```python
from build123d import *

# Parameters (mm, degrees)
SKETCH_1_R          = 52.5
SKETCH_1_R_2        = 16
SKETCH_1_R_3        = 3
EXTRUDE_1_DEPTH     = 10
SKETCH_2_R          = 24
SKETCH_2_R_2        = 16
EXTRUDE_2_DEPTH     = 20
CUT_EXTRUDE_START   = -3
CUT_EXTRUDE_2_DEPTH = 3


with BuildPart() as part:
    # 草图1 → 凸台-拉伸1 (new body)
    with BuildSketch(Plane.XY):
        Circle(SKETCH_1_R)
        Circle(SKETCH_1_R_2, mode=Mode.SUBTRACT)
        with Locations((0, 40)):
            Circle(SKETCH_1_R_3, mode=Mode.SUBTRACT)
        with Locations((40, 0)):
            Circle(SKETCH_1_R_3, mode=Mode.SUBTRACT)
        with Locations((0, -40)):
            Circle(SKETCH_1_R_3, mode=Mode.SUBTRACT)
        with Locations((-40, 0)):
            Circle(SKETCH_1_R_3, mode=Mode.SUBTRACT)
    extrude(amount=EXTRUDE_1_DEPTH)

    # 草图2 → 凸台-拉伸2 (add)
    with BuildSketch(Plane.XY.offset(10)):
        Circle(SKETCH_2_R)
        Circle(SKETCH_2_R_2, mode=Mode.SUBTRACT)
    extrude(amount=EXTRUDE_2_DEPTH)

    # 草图3 → 切除-拉伸2 (cut)
    with BuildSketch(Plane.XY.offset(30).offset(CUT_EXTRUDE_START)):
        with BuildLine():
            Line((-4, 23.664319132), (-4, 15.491933385))
            ThreePointArc((-4, 15.491933385), (0, 16), (4, 15.491933385))
            Line((4, 15.491933385), (4, 23.664319132))
            ThreePointArc((4, 23.664319132), (0, 24), (-4, 23.664319132))
        make_face()
        with BuildLine():
            Line((13.904773406, 19.561627655), (8.126024025, 13.782878275))
            ThreePointArc((8.126024025, 13.782878275), (11.313708499, 11.313708499), (13.782878275, 8.126024025))
            Line((13.782878275, 8.126024025), (19.561627655, 13.904773406))
            ThreePointArc((19.561627655, 13.904773406), (16.970562748, 16.970562748), (13.904773406, 19.561627655))
        make_face()
        with BuildLine():
            Line((23.664319132, 4), (15.491933385, 4))
            ThreePointArc((15.491933385, 4), (16, 0), (15.491933385, -4))
            Line((15.491933385, -4), (23.664319132, -4))
            ThreePointArc((23.664319132, -4), (24, 0), (23.664319132, 4))
        make_face()
        with BuildLine():
            Line((19.561627655, -13.904773406), (13.782878275, -8.126024025))
            ThreePointArc((13.782878275, -8.126024025), (11.313708499, -11.313708499), (8.126024025, -13.782878275))
            Line((8.126024025, -13.782878275), (13.904773406, -19.561627655))
            ThreePointArc((13.904773406, -19.561627655), (16.970562748, -16.970562748), (19.561627655, -13.904773406))
        make_face()
        with BuildLine():
            Line((4, -23.664319132), (4, -15.491933385))
            ThreePointArc((4, -15.491933385), (0, -16), (-4, -15.491933385))
            Line((-4, -15.491933385), (-4, -23.664319132))
            ThreePointArc((-4, -23.664319132), (0, -24), (4, -23.664319132))
        make_face()
        with BuildLine():
            Line((-13.904773406, -19.561627655), (-8.126024025, -13.782878275))
            ThreePointArc((-8.126024025, -13.782878275), (-11.313708499, -11.313708499), (-13.782878275, -8.126024025))
            Line((-13.782878275, -8.126024025), (-19.561627655, -13.904773406))
            ThreePointArc((-19.561627655, -13.904773406), (-16.970562748, -16.970562748), (-13.904773406, -19.561627655))
        make_face()
        with BuildLine():
            Line((-23.664319132, -4), (-15.491933385, -4))
            ThreePointArc((-15.491933385, -4), (-16, 0), (-15.491933385, 4))
            Line((-15.491933385, 4), (-23.664319132, 4))
            ThreePointArc((-23.664319132, 4), (-24, 0), (-23.664319132, -4))
        make_face()
        with BuildLine():
            Line((-19.561627655, 13.904773406), (-13.782878275, 8.126024025))
            ThreePointArc((-13.782878275, 8.126024025), (-11.313708499, 11.313708499), (-8.126024025, 13.782878275))
            Line((-8.126024025, 13.782878275), (-13.904773406, 19.561627655))
            ThreePointArc((-13.904773406, 19.561627655), (-16.970562748, 16.970562748), (-19.561627655, 13.904773406))
        make_face()
    extrude(amount=CUT_EXTRUDE_2_DEPTH, mode=Mode.SUBTRACT)


solid = part.part
```
Part model, mm, in its own coordinate system. A direction names the side the tool comes from. Coordinates: 2 decimals unless noted, no trailing zeros. Loops run counter-clockwise (first coordinate to the right, second up) from the corner with the lowest first, then second, coordinate; pieces in that order, holes last. Notation, with made-up numbers: (5, 55) - (23, 55) arc R28 cw to (23, 81) - close; hole circle Ø6 at (-10, -1). An arc over 180 degrees is marked (long way). Write item = value, one per line. Start each with the question number.
Item 1: Cut at C-C, the plane z = 2.25. Give the cut face in (x, y).
Item 2: Wall check: L1, parallel to Y at x = 0, z = 2.5; L2, parallel to Y at x = 0, z = 12.75; L3, parallel to Z at x = 17.5, y = 34.5. Give the ranges that are in metal, low to high. Write a range as from..to.
Item 3: Cut at D-D, the plane y = 40. Give the cut face in (x, z), and give its area (3 significant figures).
Item 4: Mould opens along X. For faces 4 (the flat face through (-19, -8, 30)), 5 (the cylindrical face through (37, 0, 5)), 6 (the cylindrical face through (50.076, 15.77, 4.93)) say: released by +X, released by -X, zero draft, split by the parting line, or undercut.
Item 5: Cut at A-A, the plane y = 0. Give the cut face in (x, z).
Item 6: 3-axis set-ups, long thin cutter, end or side, ignore diameter. For faces 1 (the flat face through (-4, -20, 28)), 2 (the flat face through (20, 4, 28)), 3 (the flat face through (-8, 19, 30)): which of +Z, -Z, +X, -X, +Y, -Y reach the whole face in a straight line?
Item 7: Flat gauge pins, fed straight in: pin 1 Ø8 at (y, z) = (-1, 26) entering from -X; pin 2 Ø4 at (x, y) = (18.5, 0) entering from +Z; pin 3 Ø5 at (x, y) = (23, -16) entering from +Z; pin 4 Ø8 at (x, y) = (14, 7) entering from +Z. Where does each tip first touch, or does it go through?
The answers:
q1.outline = circle Ø105 at (0, 0); hole circle Ø6 at (-40, 0); hole circle Ø32 at (0, 0); hole circle Ø6 at (0, -40); hole circle Ø6 at (0, 40); hole circle Ø6 at (40, 0)
q2.L1 = -52.5..-43, -37..-16, 16..37, 43..52.5
q2.L2 = -24..-16, 16..24
q2.L3 = 0..10
q3.outline = (-34, 0) - (-3, 0) - (-3, 10) - (-34, 10) - close; (3, 0) - (34, 0) - (34, 10) - (3, 10) - close
q3.area = 620 mm2
q4.face_4 = zero draft
q4.face_5 = undercut
q4.face_6 = split by the parting line
q5.outline = (-52.5, 0) - (-43, 0) - (-43, 10) - (-52.5, 10) - close; (-37, 0) - (-16, 0) - (-16, 27) - (-24, 27) - (-24, 10) - (-37, 10) - close; (16, 0) - (37, 0) - (37, 10) - (24, 10) - (24, 27) - (16, 27) - close; (43, 0) - (52.5, 0) - (52.5, 10) - (43, 10) - close
q6.face_1 = +Z, +Y, -Y
q6.face_2 = +Z, +X, -X
q6.face_3 = +Z, +X, -X, +Y, -Y
q7.pin_1 = -24
q7.pin_2 = 27
q7.pin_3 = 10
q7.pin_4 = 30
